from build123d import *

# Parameters (mm, degrees)
CHAMFER_1_SIZE      = 0.5
CUT_EXTRUDE_START   = -11
CUT_EXTRUDE_1_DEPTH = 10


with BuildPart() as part:
    # 草图1 → 旋转1 (revolve)
    with BuildSketch(Plane(origin=(0, 0, 0), x_dir=(-1, 0, 0), z_dir=(0, 0, -1)), mode=Mode.PRIVATE) as revolve_1_sk:
        Polygon((-60, 17.5), (60, 17.5), (60, 15), (93, 15), (93, 12.5), (138, 12.5), (138, 0), (-138, 0), (-138, 12.5), (-93, 12.5), (-93, 15), (-60, 15), align=None)
    revolve(revolve_1_sk.sketch.rotate(Axis((70, 0, 0), (-1, 0, 0)), 270), axis=Axis((70, 0, 0), (-1, 0, 0)))

    # 倒角1
    chamfer_1_edges = [part.edges().sort_by_distance(p)[0] for p in [
        (-138, 0, -12.5),
        (-93, 0, -15),
        (-60, 0, -17.5),
        (60, 0, -17.5),
        (93, 0, -15),
    ]]
    chamfer(chamfer_1_edges, length=CHAMFER_1_SIZE)

    # 草图2 → 切除-拉伸1 (cut)
    with BuildSketch(Plane.XY.offset(CUT_EXTRUDE_START)):
        with BuildLine():
            Line((-77, 4), (-65, 4))
            ThreePointArc((-65, 4), (-61, 0), (-65, -4))
            Line((-65, -4), (-77, -4))
            ThreePointArc((-77, -4), (-81, 0), (-77, 4))
        make_face()
        with BuildLine():
            Line((65, 4), (77, 4))
            ThreePointArc((77, 4), (81, 0), (77, -4))
            Line((77, -4), (65, -4))
            ThreePointArc((65, -4), (61, 0), (65, 4))
        make_face()
    extrude(amount=-CUT_EXTRUDE_1_DEPTH, mode=Mode.SUBTRACT)


solid = part.part
The listing builds one solid part. Answer for the finished solid, in the listing's coordinates (mm). A direction names the side the tool comes from. Coordinates: 2 decimals unless noted, no trailing zeros. Order: outer loops, then holes, each group sorted by start corner. A loop starts at its lowest first (then second) coordinate and runs counter-clockwise, first axis right, second up. Notation, with made-up numbers: (1, 10) -> (49, 10) arc R23 cw to (49, 46) -> close; hole circle Ø1 at (22.5, 69). An arc over 180 degrees is marked (long way). Answer in a Markdown table with one row per item. Add a question column.
Item 1: Find the intervals of material crossed by L1, parallel to X at y = 14, z = -1.5; L2, parallel to Y at x = 38, z = 0; L3, parallel to Y at x = 69, z = -1, in increasing order. Write a range as from..to.
Item 2: Find section D-D (x = -110). Write down the section's boundary in (y, z).
Item 3: Find section B-B (x = -70). Write down the section's boundary in (y, z).
Item 4: Determine the mould class of faces 4 (the face through (71, 0, -11)), 5 (the face through (-71, 0, -11)), 6 (the face through (-60, -14, 6)), 7 (the face through (-115.562, 3.755, 11.923)) for opening direction X: +X half, -X half, draft (parallel to the pull), parting line (faces both ways), or undercut.
Item 5: Find section C-C (x = 51.5). Write down the section's boundary in (y, z).
Item 6: Which of the six approach directions +Z, -Z, +X, -X, +Y, -Y give full straight-line access (tool end or side, diameter ignored) to faces 1 (the face through (-93, 7, -11)), 2 (the face through (-0.833, -10.648, -13.887)), 3 (the face through (115.185, 3.755, 11.923))?
Item 7: Each of these flat-tipped pins is pushed along its axis until it touches: P1, Ø4, axis at x = -71, y = 1, coming from the -Z side; P2, Ø1, axis at x = -39.5, y = 7.5, coming from the -Z side; P3, Ø12, axis at x = -87.5, z = 0.5, coming from the +Y side; P4, Ø5, axis at y = 12, z = 4, coming from the +X side. Where does it stop, or does it pass through?
Result set:
| question | item | result |
|---|---|---|
| 1 | L1 | x = -93..93 |
| 1 | L2 | y = -17.5..17.5 |
| 1 | L3 | y = -14.97..14.97 |
| 2 | outline | circle Ø25 at (0, 0) |
| 3 | outline | (-4, -14.46) -> (-4, -11) -> (4, -11) -> (4, -14.46) arc R15 ccw (long way) to start |
| 4 | face 4 | undercut |
| 4 | face 5 | undercut |
| 4 | face 6 | -X half |
| 4 | face 7 | draft |
| 5 | outline | circle Ø35 at (0, 0) |
| 6 | face 1 | -X |
| 6 | face 2 | +X, -X |
| 6 | face 3 | +X |
| 7 | P1 | stops at z = -11 |
| 7 | P2 | stops at z = -16.04 |
| 7 | P3 | stops at y = 15 |
| 7 | P4 | stops at x = 138 |
